Source: CAD feature listing. Evaluate the final solid. Frame: model axes, mm. A direction names the side the tool comes from. Give positions to 0.01 mm unless a question says otherwise; leave off trailing zeros. Order: outer loops, then holes, each group sorted by start corner. A loop starts at its lowest first (then second) coordinate and runs counter-clockwise, first axis right, second up.
from build123d import *

# Parameters (mm, degrees)
BOSS_EXTRUDE1_DEPTH     = 55
SKETCH2_W               = 60
SKETCH2_H               = 2
CUT_EXTRUDE1_DEPTH      = 212
SKETCH3_R               = 16
BOSS_EXTRUDE2_DEPTH     = 3
SKETCH4_R               = 12.5
CUT_EXTRUDE2_DEPTH      = 56
SKETCH5_R               = 12.5
BOSS_EXTRUDE3_DEPTH     = 3
SKETCH6_R               = 8.5
CUT_EXTRUDE3_DEPTH      = 66
CUT_EXTRUDE4_DEPTH      = 28
SKETCH9_R               = 6.5
BOSS_EXTRUDE4_DEPTH     = 22
FILLET1_R               = 10
CUT_EXTRUDE5_DEPTH      = 15.5
CUT_EXTRUDE5_DEPTH_BACK = 1.5
SKETCH10_R              = 15
SKETCH12_W              = 110
SKETCH12_H              = 12.5
SKETCH12_H_2            = 2.5
SKETCH12_H_3            = 10
SKETCH12_W_2            = 15
CUT_EXTRUDE7_DEPTH      = 12
SKETCH13_R              = 3
CUT_EXTRUDE8_DEPTH      = 10


with BuildPart() as part:
    # Sketch1 → Boss-Extrude1 (new, symmetric)
    with BuildSketch(Plane.XY):
        Polygon((0, 0), (194, 0), (194, 29.332947361), (194, 76), (172, 76), (172, 50), (164, 50), (164, 40), (0, 40), align=None)
    extrude(amount=BOSS_EXTRUDE1_DEPTH, both=True)

    # Sketch2 → Cut-Extrude1 (cut)
    with BuildSketch(Plane(origin=(194, 0, 0), x_dir=(0, 0, -1), z_dir=(1, 0, 0))):
        with Locations((0, 1)):
            Rectangle(SKETCH2_W, SKETCH2_H)
    extrude(amount=-CUT_EXTRUDE1_DEPTH, mode=Mode.SUBTRACT)

    # Sketch3 → Boss-Extrude2 (add)
    with BuildSketch(Plane(origin=(194, 0, 0), x_dir=(0, 0, -1), z_dir=(1, 0, 0))):
        with Locations(Location((0, 18, 0), (0, 0, 270))):
            Circle(SKETCH3_R)
    extrude(amount=BOSS_EXTRUDE2_DEPTH)

    # Sketch4 → Cut-Extrude2 (cut)
    with BuildSketch(Plane(origin=(197, 0, 0), x_dir=(0, 0, -1), z_dir=(1, 0, 0))):
        with Locations((0, 18)):
            Circle(SKETCH4_R)
    extrude(amount=-CUT_EXTRUDE2_DEPTH, mode=Mode.SUBTRACT)

    # Sketch5 → Boss-Extrude3 (add)
    with BuildSketch(Plane.ZY):
        with Locations(Location((0, 18, 0), (0, 0, 180))):
            Circle(SKETCH5_R)
    extrude(amount=BOSS_EXTRUDE3_DEPTH)

    # Sketch6 → Cut-Extrude3 (cut)
    with BuildSketch(Plane.ZY.offset(3)):
        with Locations(Location((0, 18, 0), (0, 0, 270))):
            Circle(SKETCH6_R)
    extrude(amount=-CUT_EXTRUDE3_DEPTH, mode=Mode.SUBTRACT)

    # Sketch7 → Cut-Extrude4 (cut)
    with BuildSketch(Plane(origin=(0, 40, 0), x_dir=(1, 0, 0), z_dir=(0, 1, 0))):
        Polygon((164, 32.5), (149, 32.5), (149, 20), (39, 20), (39, 32.5), (24, 32.5), (24, -32.5), (39, -32.5), (39, -20), (149, -20), (149, -32.5), (164, -32.5), align=None)
    extrude(amount=-CUT_EXTRUDE4_DEPTH, mode=Mode.SUBTRACT)

    # Sketch9 → Boss-Extrude4 (add)
    with BuildSketch(Plane.XZ):
        with BuildLine():
            Line((117, 75), (117, 65))
            ThreePointArc((117, 65), (119.928932188, 57.928932188), (127, 55))
            Line((127, 55), (67, 55))
            ThreePointArc((67, 55), (74.071067812, 57.928932188), (77, 65))
            Line((77, 65), (77, 75))
            ThreePointArc((77, 75), (97, 95), (117, 75))
        make_face()
        with Locations(Location((97, 75, 0), (0, 0, 270))):
            Circle(SKETCH9_R, mode=Mode.SUBTRACT)
    extrude(amount=-BOSS_EXTRUDE4_DEPTH)

    # Fillet1
    fillet1_edges = [part.edges().sort_by_distance(p)[0] for p in [
        (97, 22, 55),
    ]]
    fillet(fillet1_edges, radius=FILLET1_R)

    # Sketch10 → Cut-Extrude5 (cut, two sides: drawn at the far end of the back side and taken through both)
    with BuildSketch(Plane(origin=(0, 22, 0), x_dir=(1, 0, 0), z_dir=(0, 1, 0)).offset(-CUT_EXTRUDE5_DEPTH_BACK)):
        with Locations(Location((97, -75, 0), (0, 0, 138.189685104))):
            Circle(SKETCH10_R)
    extrude(amount=CUT_EXTRUDE5_DEPTH + CUT_EXTRUDE5_DEPTH_BACK, mode=Mode.SUBTRACT)

    # Mirror17: part across plane


with BuildPart() as part_1:
    add(part.part)
    add(part.part.mirror(Plane.XY))

    # Sketch12 → Cut-Extrude7 (cut)
    with BuildSketch(Plane.XZ):
        Polygon((149, 20), (39, 20), (39, 32.5), (24, 32.5), (24, -30), (39, -30), (39, -20), (149, -20), (149, -30), (164, -30), (164, 32.5), (149, 32.5), align=None)
        with Locations((94, 26.25)):
            Rectangle(SKETCH12_W, SKETCH12_H)
        with Locations((94, -31.25)):
            Rectangle(SKETCH12_W, SKETCH12_H_2)
        with Locations((94, -25)):
            Rectangle(SKETCH12_W, SKETCH12_H_3)
        with Locations((31.5, -31.25)):
            Rectangle(SKETCH12_W_2, SKETCH12_H_2)
        with Locations((156.5, -31.25)):
            Rectangle(SKETCH12_W_2, SKETCH12_H_2)
    extrude(amount=-CUT_EXTRUDE7_DEPTH, mode=Mode.SUBTRACT)

    # Sketch13 → Cut-Extrude8 (cut)
    with BuildSketch(Plane.ZY.offset(-172)):
        with Locations(Location((38, 63, 0), (0, 0, 270))):
            Circle(SKETCH13_R)
        with Locations(Location((-38, 63, 0), (0, 0, 90))):
            Circle(SKETCH13_R)
    extrude(amount=-CUT_EXTRUDE8_DEPTH, mode=Mode.SUBTRACT)


solid = part_1.part
1) Ray query, L1, parallel to Z at x = 97, y = 21; L2, parallel to Z at x = 179.25, y = 63; L3, parallel to X at y = 19.5, z = -27.5. Return the intervals inside material, ascending.
Checks:
L1: z = -95 to -90, -60 to -20, 20 to 60, 90 to 95
L2: z = -55 to -41, -35 to 35, 41 to 55
L3: x = 0 to 24, 39 to 149, 164 to 194
2) Pull-direction query (X, two-part tool) for faces 1 (the face through (95, 11, 32.5)), 2 (the face through (182, 63, 38)), 3 (the face through (12, 2, 0)); classes: +X half, -X half, draft (parallel to the pull), parting line (faces both ways), or undercut.
Checks:
face 1: undercut
face 2: -X half
face 3: draft
3) First-contact query: pin 1 Ø6 at (y, z) = (23, 25.5) entering from +X; pin 2 Ø5 at (y, z) = (65.5, 3.5) entering from -X; pin 3 Ø9 at (x, z) = (178.5, 5) entering from -Y. Flat tips, straight axial feed; report the tip coordinate or a pass-through.
Checks:
pin 1: stops at x = 194
pin 2: stops at x = 172
pin 3: stops at y = 2
4) Section query B-B on x = 97. State how many separate pieces and enclosed holes the cut face has, and give its area (3 significant figures).
Checks:
separate pieces: 4
enclosed holes: 0
area: 3,680 mm2
5) Section query A-A on x = 45.5. Output: boundary loops of the cut face in (y, z).
Checks:
outline: (0, -55) - (40, -55) - (40, -20) - (12, -20) - (12, -32.5) - (0, -32.5) - close; (0, 32.5) - (12, 32.5) - (12, 20) - (40, 20) - (40, 55) - (0, 55) - close
6) Section query D-D on x = 10.5. Output: boundary loops of the cut face in (y, z), and give its area (3 significant figures).
Checks:
outline: (0, -55) - (40, -55) - (40, 55) - (0, 55) - (0, 30) - (2, 30) - (2, -30) - (0, -30) - close; hole circle Ø17 at (18, 0)
area: 4,050 mm2
7) Section query C-C on z = -23. Output: boundary loops of the cut face in (x, y).
Checks:
outline: (0, 2) - (24, 2) - (24, 40) - (0, 40) - close; (39, 12) - (149, 12) - (149, 40) - (39, 40) - close; (164, 2) - (194, 2) - (194, 76) - (172, 76) - (172, 50) - (164, 50) - close
8) Reachability of faces 4 (the face through (95, 11, -32.5)), 5 (the face through (164, 31, 1)), 6 (the face through (195.479, 30.697, 9.736)) from +Z, -Z, +X, -X, +Y, -Y: full face, straight path, thin tool, end or side. Return the list, or none.
Checks:
face 4: -Y
face 5: +Y
face 6: +X
